Read the model definition and answer for the solid it produces. Units are mm, in the model's axes. Face numbers are marked on the shaded views. Give positions to 0.01 mm unless a question says otherwise; leave off trailing zeros. Loops run counter-clockwise (first coordinate to the right, second up) from the corner with the lowest first, then second, coordinate; pieces in that order, holes last. Notation, with made-up numbers: (-30, 87.5) - (4, 87.5) arc R30 ccw to (4, 121.5) - close; hole circle Ø11 at (-36, 45.25). An arc over 180 degrees is marked (long way). Write item = value, one per line.
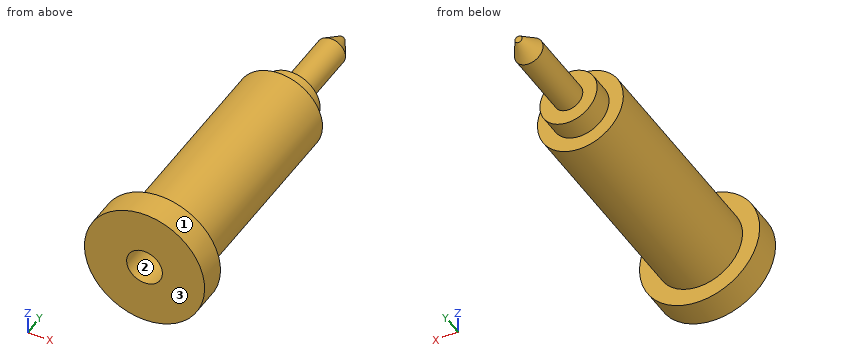
```python
from build123d import *


with BuildPart() as part:
    # Sketch1 → Revolve1 (revolve)
    with BuildSketch(Plane.XY, mode=Mode.PRIVATE) as revolve1_sk:
        Polygon((-1.25, 0), (-4.2, 0), (-4.2, 2), (-3, 2), (-3, 17), (-2, 17), (-2, 18.5), (-1, 18.5), (-1, 23.5), (-0.25, 24.799038106), (0, 24.799038106), (0, 6), (-1.25, 6), align=None)
    revolve(revolve1_sk.sketch.rotate(Axis((0, 0, 0), (0, 1, 0)), 270), axis=Axis((0, 0, 0), (0, 1, 0)))


solid = part.part
```
1) A cutting plane is placed at A-A on z = 0. Determine the outline of the cut face in (x, y), then the cut area to 3 significant figures.
Output:
outline = (-4.2, 0) - (-1.25, 0) - (-1.25, 6) - (1.25, 6) - (1.25, 0) - (4.2, 0) - (4.2, 2) - (3, 2) - (3, 17) - (2, 17) - (2, 18.5) - (1, 18.5) - (1, 23.5) - (0.25, 24.8) - (-0.25, 24.8) - (-1, 23.5) - (-1, 18.5) - (-2, 18.5) - (-2, 17) - (-3, 17) - (-3, 2) - (-4.2, 2) - close
area = 109 mm²
2) A cutting plane is placed at D-D on z = -1.75. Determine the outline of the cut face in (x, y).
Output:
outline = (-3.82, 0) - (3.82, 0) - (3.82, 2) - (2.44, 2) - (2.44, 17) - (0.97, 17) - (0.97, 18.5) - (-0.97, 18.5) - (-0.97, 17) - (-2.44, 17) - (-2.44, 2) - (-3.82, 2) - close
3) The mould has two halves that part along Z. Classify the marked faces 1, 2 and 3: pulls with the +Z half, pulls with the -Z half, needs draft (parallel to the pull), parting line crosses it, or undercut.
Output:
face_1 = parting line crosses it
face_2 = undercut
face_3 = needs draft
4) A cutting plane is placed at C-C on y = 8.75. Determine the outline of the cut face in (x, z), then the cut area to 3 significant figures.
Output:
outline = circle Ø6 at (0, 0)
area = 28.3 mm²
5) Find the intervals of material crossed by probe 1 along X at (y, z) = (4, 0); probe 2 along X at (y, z) = (1.5, 0); probe 3 along Y at (x, z) = (2.75, -0.25), in increasing order.
Output:
probe_1 = -3 to -1.25, 1.25 to 3
probe_2 = -4.2 to -1.25, 1.25 to 4.2
probe_3 = 0 to 17
6) Each of these flat-tipped pins is pushed along its axis until it touches: P1, Ø2, axis at y = 20.5, z = -3, coming from the -X side; P2, Ø1, axis at x = -1.5, y = 8.5, coming from the -Z side; P3, Ø3, axis at y = 5, z = 2, coming from the +X side. Where does it stop, or does it pass through?
Output:
P1 = through
P2 = -2.83
P3 = 2.96
7) A cutting plane is placed at B-B on x = 0. Determine the outline of the cut face in (y, z), then the cut area to 3 significant figures.
Output:
outline = (0, -4.2) - (2, -4.2) - (2, -3) - (17, -3) - (17, -2) - (18.5, -2) - (18.5, -1) - (23.5, -1) - (24.8, -0.25) - (24.8, 0.25) - (23.5, 1) - (18.5, 1) - (18.5, 2) - (17, 2) - (17, 3) - (2, 3) - (2, 4.2) - (0, 4.2) - (0, 1.25) - (6, 1.25) - (6, -1.25) - (0, -1.25) - close
area = 109 mm²
